```python
from build123d import *

# Parameters (mm, degrees)
SKETCH1_W              = 200
SKETCH1_H              = 90
BOSS_EXTRUDE1_DEPTH    = 14
M12_TAPPED_HOLE1_D     = 10.2
M12_TAPPED_HOLE1_DEPTH = 29.25
M12_TAPPED_HOLE1_TIP   = 3.064389157
FILLET1_R              = 10
M20X1_5_TAPPED_HOLE1_D = 18.5
M8_TAPPED_HOLE1_D      = 6.8


with BuildPart() as part:
    # Sketch1 → Boss-Extrude1 (new body)
    with BuildSketch(Plane(origin=(0, 0, 0), x_dir=(1, 0, 0), z_dir=(0, 1, 0))):
        with Locations((100, 45)):
            Rectangle(SKETCH1_W, SKETCH1_H)
    extrude(amount=BOSS_EXTRUDE1_DEPTH)

    # M12 Tapped Hole1
    with Locations(Plane(origin=(0, 14, 0), x_dir=(1, 0, 0), z_dir=(0, 1, 0))):
        with Locations((10, 45), (190, 45)):
            Hole(M12_TAPPED_HOLE1_D / 2, depth=M12_TAPPED_HOLE1_DEPTH)
            with Locations((0, 0, -(M12_TAPPED_HOLE1_DEPTH + M12_TAPPED_HOLE1_TIP / 2))):  # 118° drill point
                Cone(0, M12_TAPPED_HOLE1_D / 2, M12_TAPPED_HOLE1_TIP, mode=Mode.SUBTRACT)

    # Fillet1
    fillet1_edges = [part.edges().sort_by_distance(p)[0] for p in [
        (0, 7, -90),
        (200, 7, -90),
        (200, 7, 0),
        (0, 7, 0),
    ]]
    fillet(fillet1_edges, radius=FILLET1_R)

    # M20x1.5 Tapped Hole1 (through all)
    with Locations(Plane(origin=(0, 14, 0), x_dir=(1, 0, 0), z_dir=(0, 1, 0))):
        with Locations((100, 45)):
            Hole(M20X1_5_TAPPED_HOLE1_D / 2)

    # M8 Tapped Hole1 (through all)
    with Locations(Plane(origin=(0, 14, 0), x_dir=(1, 0, 0), z_dir=(0, 1, 0))):
        with Locations((20, 75), (100, 75), (180, 75), (180, 15), (100, 15), (20, 15)):
            Hole(M8_TAPPED_HOLE1_D / 2)


solid = part.part
```
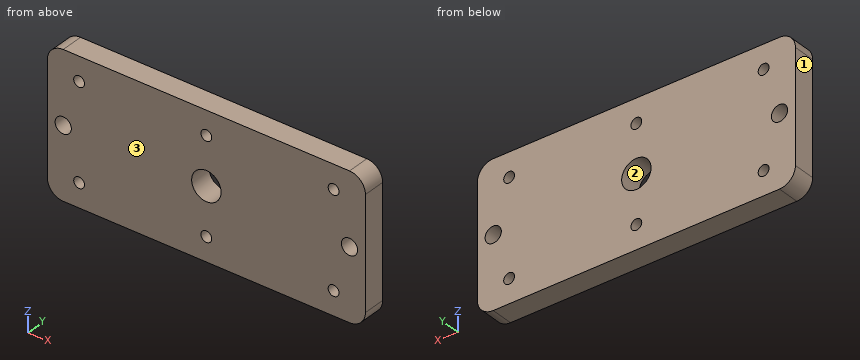
Can you work these out from the model? Positions are in its coordinate system, mm. Face numbers are marked on the shaded views. Coordinates: 2 decimals unless noted, no trailing zeros. Loops run counter-clockwise (first coordinate to the right, second up) from the corner with the lowest first, then second, coordinate; pieces in that order, holes last.
1) Imagine slicing it at A-A on x = 100. List the corners of the cut face in (y, z) for me, plus the area to 3 significant figures.
2) Thinking about a two-plate mould opening in X: for the marked faces 1, 2 and 3, which applies, pulls with the +X half, pulls with the -X half, needs draft (parallel to the pull), parting line crosses it, or undercut?
3) I need wall thicknesses on probe 1 along X at (y, z) = (10, -15); probe 2 along Z at (x, y) = (20, 5.25); probe 3 along X at (y, z) = (4.5, -45). Which ranges of each line are inside material? Lowest first, please.
4) Imagine slicing it at C-C on z = -45. List the corners of the cut face in (x, y) for me, plus the area to 3 significant figures.
5) Imagine slicing it at D-D on x = 20. List the corners of the cut face in (y, z) for me, plus the area to 3 significant figures.
6) Imagine slicing it at B-B on y = 3.5. State how many separate pieces and enclosed holes the cut face has, plus the area to 3 significant figures.
Completed:
1. outline: (0, -90) - (14, -90) - (14, -78.4) - (0, -78.4) - close; (0, -71.6) - (14, -71.6) - (14, -54.25) - (0, -54.25) - close; (0, -35.75) - (14, -35.75) - (14, -18.4) - (0, -18.4) - close; (0, -11.6) - (14, -11.6) - (14, 0) - (0, 0) - close
1. area: 811 mm2
2. face 1: pulls with the -X half
2. face 2: undercut
2. face 3: needs draft
3. probe 1: x = 0 to 16.6, 23.4 to 96.6, 103.4 to 176.6, 183.4 to 200
3. probe 2: z = -90 to -78.4, -71.6 to -18.4, -11.6 to 0
3. probe 3: x = 0 to 4.9, 15.1 to 90.75, 109.25 to 184.9, 195.1 to 200
4. outline: (0, 0) - (4.9, 0) - (4.9, 14) - (0, 14) - close; (15.1, 0) - (90.75, 0) - (90.75, 14) - (15.1, 14) - close; (109.25, 0) - (184.9, 0) - (184.9, 14) - (109.25, 14) - close; (195.1, 0) - (200, 0) - (200, 14) - (195.1, 14) - close
4. area: 2,260 mm2
5. outline: (0, -90) - (14, -90) - (14, -78.4) - (0, -78.4) - close; (0, -71.6) - (14, -71.6) - (14, -18.4) - (0, -18.4) - close; (0, -11.6) - (14, -11.6) - (14, 0) - (0, 0) - close
5. area: 1,070 mm2
6. separate pieces: 1
6. enclosed holes: 9
6. area: 17,300 mm2
